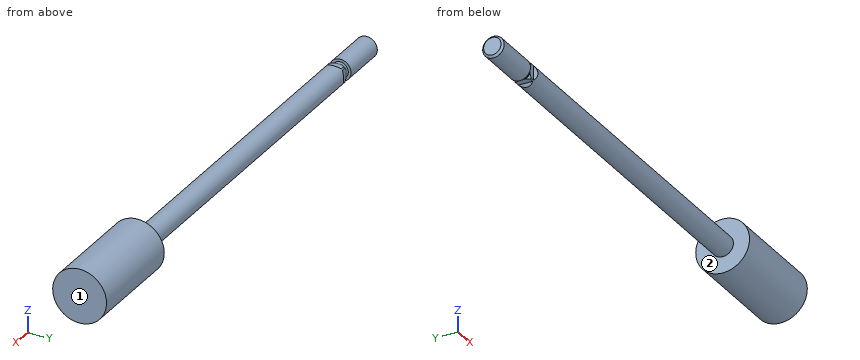
from build123d import *

# Parameters (mm, degrees)
CUT_EXTRUDE_1_DEPTH      = 4
CUT_EXTRUDE_1_DEPTH_BACK = 4
CUT_EXTRUDE_2_DEPTH      = 4
CUT_EXTRUDE_2_DEPTH_BACK = 4
CUT_EXTRUDE_3_DEPTH      = 4
CUT_EXTRUDE_3_DEPTH_BACK = 4
CUT_EXTRUDE_4_DEPTH      = 4
CUT_EXTRUDE_4_DEPTH_BACK = 4
SCALE_1_SCALE            = 0.5


with BuildPart() as part:
    # 草图1 → 旋转1 (revolve)
    with BuildSketch(Plane.XY, mode=Mode.PRIVATE) as revolve_1_sk:
        Polygon((-40, 0), (-40, 3.233), (-39.233, 4), (-21.5, 4), (-21.5, 3), (-20, 3), (-20, 3.25), (-19.25, 4), (115.5, 4), (115.5, 10), (154.5, 10), (154.5, 0), align=None)
    revolve(revolve_1_sk.sketch.rotate(Axis((154.5, 0, 0), (-1, 0, 0)), 270), axis=Axis((154.5, 0, 0), (-1, 0, 0)))

    # 草图2 → 切除-拉伸1 (cut, two sides: drawn at the far end of the back side and taken through both)
    with BuildSketch(Plane.XY.offset(-CUT_EXTRUDE_1_DEPTH_BACK)):
        Polygon((-20, 3), (-17.5, 3), (-16.5, 4), (-20, 4), align=None)
    extrude(amount=CUT_EXTRUDE_1_DEPTH + CUT_EXTRUDE_1_DEPTH_BACK, mode=Mode.SUBTRACT)

    # 草图3 → 切除-拉伸2 (cut, two sides: drawn at the far end of the back side and taken through both)
    with BuildSketch(Plane.XY.offset(-CUT_EXTRUDE_2_DEPTH_BACK)):
        Polygon((-20, -3), (-20, -4), (-16.5, -4), (-17.5, -3), align=None)
    extrude(amount=CUT_EXTRUDE_2_DEPTH + CUT_EXTRUDE_2_DEPTH_BACK, mode=Mode.SUBTRACT)

    # 草图4 → 切除-拉伸3 (cut, two sides: drawn at the far end of the back side and taken through both)
    with BuildSketch(Plane(origin=(0, 0, 0), x_dir=(1, 0, 0), z_dir=(0, 1, 0)).offset(-CUT_EXTRUDE_3_DEPTH_BACK)):
        Polygon((-20, 3), (-17.5, 3), (-16.5, 4), (-20, 4), align=None)
    extrude(amount=CUT_EXTRUDE_3_DEPTH + CUT_EXTRUDE_3_DEPTH_BACK, mode=Mode.SUBTRACT)

    # 草图5 → 切除-拉伸4 (cut, two sides: drawn at the far end of the back side and taken through both)
    with BuildSketch(Plane(origin=(0, 0, 0), x_dir=(1, 0, 0), z_dir=(0, 1, 0)).offset(-CUT_EXTRUDE_4_DEPTH_BACK)):
        Polygon((-20, -3), (-20, -4), (-16.5, -4), (-17.5, -3), align=None)
    extrude(amount=CUT_EXTRUDE_4_DEPTH + CUT_EXTRUDE_4_DEPTH_BACK, mode=Mode.SUBTRACT)


with BuildPart() as part_1:
    # 缩放比例1: scaled about (97.615985287, 0, 0)
    add(part.part.scale(SCALE_1_SCALE).moved(Location((48.807992644, 0, 0))))


solid = part_1.part
Work out the finished part from the listing and answer in its coordinate system (mm). Face numbers are marked on the shaded views. A direction names the side the tool comes from. Round coordinates to 2 decimals unless told otherwise and drop trailing zeros. Write each loop counter-clockwise with the first axis right and the second up, starting at its lowest first coordinate (ties: lowest second). Pieces come first, ordered by that corner, then holes. Notation, with made-up numbers: (1, -0.75) - (46, -0.75) arc R11 cw to (46, 6.25) - close; hole circle Ø4 at (51.25, 26.25). An arc over 180 degrees is marked (long way). Answer in a Markdown table with one row per item. Add a question column.
1. For the marked faces 1 and 2, determine the directions among +Z, -Z, +X, -X, +Y, -Y from which every point of the face is accessible in a straight line to the end or side of a thin tool.
2. A cutting plane is placed at C-C, the plane y = 3.5. Determine the outline of the cut face in (x, z), and give its area (3 significant figures).
3. A cutting plane is placed at A-A, the plane x = 84. Determine the outline of the cut face in (y, z).
4. Find the intervals of material crossed by line 1 along X through (y, z) = (3.25, 0); line 2 along Z through (x, y) = (63.5, -0.25); line 3 along Y through (x, z) = (66.5, 1.5), in increasing order. Write a range as from..to.
5. A cutting plane is placed at B-B, the plane z = 4. Determine the outline of the cut face in (x, y), and give its area (3 significant figures).
6. Given pin 1 (1 mm diameter, centred on x = 39.5, y = 0, fed in from +Z); pin 2 (3 mm diameter, centred on y = -1.5, z = -3, fed in from -X); pin 3 (3 mm diameter, centred on x = 77.5, y = -1, fed in from -Z), each flat-ended and moving along its own axis, determine where each tip first touches the part or whether it passes through.
Worked out:
| question | item | result |
|---|---|---|
| 1 | face 1 | +Z, -Z, +X, +Y, -Y |
| 1 | face 2 | -X |
| 2 | outline | (106.56, -3.57) - (126.06, -3.57) - (126.06, 3.57) - (106.56, 3.57) - close |
| 2 | area | 139 mm^2 |
| 3 | outline | circle Ø4 at (0, 0) |
| 4 | line 1 | 106.56..126.06 |
| 4 | line 2 | -1.98..1.98 |
| 4 | line 3 | -1.32..1.32 |
| 5 | outline | (106.56, -3) - (126.06, -3) - (126.06, 3) - (106.56, 3) - close |
| 5 | area | 117 mm^2 |
| 6 | pin 1 | z = 1.5 |
| 6 | pin 2 | x = 29.05 |
| 6 | pin 3 | z = -2 |
